Geometry: final body of the model. Coordinates: model frame, mm. A direction names the side the tool comes from. Round coordinates to 2 decimals unless told otherwise and drop trailing zeros. Write each loop counter-clockwise with the first axis right and the second up, starting at its lowest first coordinate (ties: lowest second). Pieces come first, ordered by that corner, then holes. Notation, with made-up numbers: (75.5, -36) -> (130.5, -36) arc R20 ccw to (130.5, -16) -> close; hole circle Ø1 at (11.25, 35). An arc over 180 degrees is marked (long way). Use one line per item in the form item = value. Start each with the question number.
1. Pin query (flat end, axial travel): pin 1 Ø6 at (x, y) = (2, 26.5) entering from +Z; pin 2 Ø4 at (x, z) = (-9, -4.5) entering from -Y; pin 3 Ø9 at (x, y) = (-19.5, 2) entering from -Z. Return the tip coordinate at first contact, or that it passes through.
2. Line query: L1, parallel to Y at x = 0, z = 7; L2, parallel to X at y = -4.5, z = 5; L3, parallel to Y at x = -1.5, z = 4.25. Output: solid intervals per line, ascending.
3. Cut plane A-A, the plane x = 0. Return the cut outline in (y, z).
4. Draft query along X for faces 4 (the face through (2, -5, -12)), 5 (the face through (-23, 0, 3)), 6 (the face through (-28, -21, 0)). Return one class per face: pulls with the +X half, pulls with the -X half, needs draft (parallel to the pull), parting line crosses it, or undercut.
5. Reachability of faces 1 (the face through (16.29, 19.12, 3.01)), 2 (the face through (23.2, -23.2, -12)), 3 (the face through (-2.38, -10.74, -8.06)) from +Z, -Z, +X, -X, +Y, -Y: full face, straight path, thin tool, end or side. Return the list, or none.
```python
from build123d import *

# Parameters (mm, degrees)
SKETCH1_R           = 35
BOSS_EXTRUDE1_DEPTH = 12
SKETCH2_R           = 5
CUT_EXTRUDE1_DEPTH  = 70.5
SKETCH3_R           = 32
SKETCH3_R_2         = 11
CUT_EXTRUDE2_DEPTH  = 8
CUT_EXTRUDE3_DEPTH  = 2
CHAMFER1_SIZE       = 0.5


with BuildPart() as part:
    # Sketch1 → Boss-Extrude1 (new, symmetric)
    with BuildSketch(Plane.XY):
        Circle(SKETCH1_R)
    extrude(amount=BOSS_EXTRUDE1_DEPTH, both=True)

    # Sketch2 → Cut-Extrude1 (cut, symmetric)
    with BuildSketch(Plane.XY.offset(12)):
        Circle(SKETCH2_R)
    extrude(amount=CUT_EXTRUDE1_DEPTH, both=True, mode=Mode.SUBTRACT)

    # Sketch3 → Cut-Extrude2 (cut)
    with BuildSketch(Plane.XY.offset(12)):
        Circle(SKETCH3_R)
        Circle(SKETCH3_R_2, mode=Mode.SUBTRACT)
    cut_extrude2 = extrude(amount=-CUT_EXTRUDE2_DEPTH, mode=Mode.SUBTRACT)

    # Mirror1: Cut-Extrude2 across plane
    add(cut_extrude2.mirror(Plane.XY), mode=Mode.SUBTRACT)

    # Sketch4 → Cut-Extrude3 (cut)
    with BuildSketch(Plane(origin=(0, 0, -4), x_dir=(-1, 0, 0), z_dir=(0, 0, -1))):
        with BuildLine():
            ThreePointArc((19.091883092, -19.091883092), (27, 0), (19.091883092, 19.091883092))
            ThreePointArc((19.091883092, 19.091883092), (16.263455967, 19.091883092), (16.263455967, 16.263455967))
            ThreePointArc((16.263455967, 16.263455967), (23, 0), (16.263455967, -16.263455967))
            ThreePointArc((16.263455967, -16.263455967), (16.263455967, -19.091883092), (19.091883092, -19.091883092))
        make_face()
        with BuildLine():
            ThreePointArc((-19.091883092, -19.091883092), (-27, 0), (-19.091883092, 19.091883092))
            ThreePointArc((-19.091883092, 19.091883092), (-16.263455967, 19.091883092), (-16.263455967, 16.263455967))
            ThreePointArc((-16.263455967, 16.263455967), (-23, 0), (-16.263455967, -16.263455967))
            ThreePointArc((-16.263455967, -16.263455967), (-16.263455967, -19.091883092), (-19.091883092, -19.091883092))
        make_face()
    cut_extrude3 = extrude(amount=-CUT_EXTRUDE3_DEPTH, mode=Mode.SUBTRACT)

    # Mirror2: Cut-Extrude3 across plane
    add(cut_extrude3.mirror(Plane.XY), mode=Mode.SUBTRACT)

    # Chamfer1
    chamfer1_edges = [part.edges().sort_by_distance(p)[0] for p in [
        (-32, 0, 12),
        (-32, 0, -12),
    ]]
    chamfer(chamfer1_edges, length=CHAMFER1_SIZE)


solid = part.part
```
Outcome:
q1.pin_1 = 4
q1.pin_2 = -34.29
q1.pin_3 = -4
q2.L1 = -35 to -32, -11 to -5, 5 to 11, 32 to 35
q2.L2 = -34.71 to -31.68, -10.04 to -2.18, 2.18 to 10.04, 31.68 to 34.71
q2.L3 = -34.97 to -31.96, -10.9 to -4.77, 4.77 to 10.9, 31.96 to 34.97
q3.outline = (-35, -12) -> (-32.5, -12) -> (-32, -11.5) -> (-32, -4) -> (-11, -4) -> (-11, -12) -> (-5, -12) -> (-5, 12) -> (-11, 12) -> (-11, 4) -> (-32, 4) -> (-32, 11.5) -> (-32.5, 12) -> (-35, 12) -> close; (5, -12) -> (11, -12) -> (11, -4) -> (32, -4) -> (32, -11.5) -> (32.5, -12) -> (35, -12) -> (35, 12) -> (32.5, 12) -> (32, 11.5) -> (32, 4) -> (11, 4) -> (11, 12) -> (5, 12) -> close
q4.face_4 = needs draft
q4.face_5 = undercut
q4.face_6 = parting line crosses it
q5.face_1 = +Z
q5.face_2 = -Z, +X, -X, +Y, -Y
q5.face_3 = -Z
